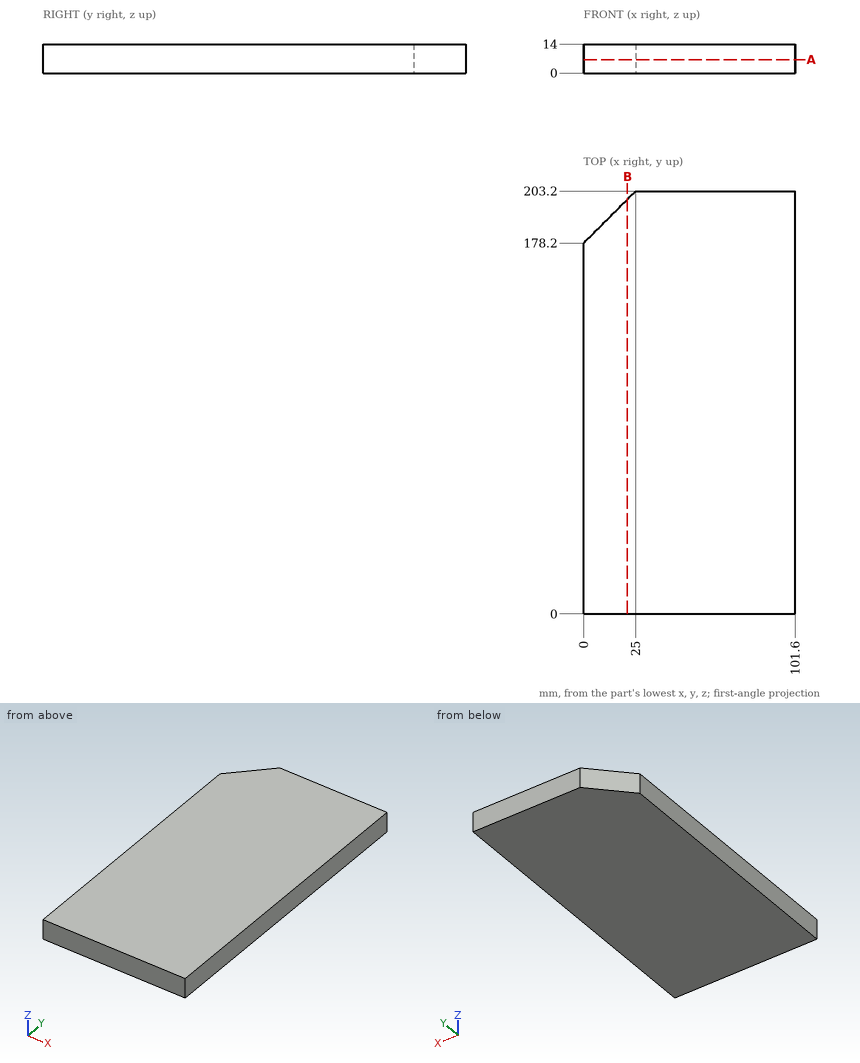
Job drawing, mm, ordinate dimensions from the low corner. One solid piece. Round coordinates to 2 decimals unless told otherwise and drop trailing zeros. Loops run counter-clockwise (first coordinate to the right, second up) from the corner with the lowest first, then second, coordinate; pieces in that order, holes last. Notation, with made-up numbers: M 15.25,55.25 L 22.25,55.25 A20 ccw 22.25,92.25 Z; hole C -34,28 d2. An arc over 180 degrees is marked long. One line per question, with ' | ' between items. Start each with the question number.
Item 1: Wall check: line 1 (X direction, y = 182.5, z = 11); line 2 (X direction, y = 183, z = 4); line 3 (Y direction, x = 16, z = 12.5). Give the ranges that are in metal, low to high.
Item 2: Cut at A-A, the plane z = 6.5. Write the cut outline in (x, y), plus the area to 3 significant figures.
Item 3: Cut at B-B, the plane x = 21. Write the cut outline in (y, z), plus the area to 3 significant figures.
Responses:
1) line 1: x = 4.3 to 101.6 | line 2: x = 4.8 to 101.6 | line 3: y = 0 to 194.2
2) outline: M 0,0 L 101.6,0 L 101.6,203.2 L 25,203.2 L 0,178.2 Z | area: 20,300 mm²
3) outline: M 0,0 L 199.2,0 L 199.2,14 L 0,14 Z | area: 2,790 mm²
